For this review, use the dimensioned drawing (mm, ordinates from the lowest corner) and the shaded views. Coordinates: 2 decimals unless noted, no trailing zeros. Write each loop counter-clockwise with the first axis right and the second up, starting at its lowest first coordinate (ties: lowest second). Pieces come first, ordered by that corner, then holes. Notation, with made-up numbers: (-8.75, 46.5) - (44.25, 46.5) arc R21 ccw to (44.25, 64.5) - close; hole circle Ø8 at (81.5, 51). An arc over 180 degrees is marked (long way). Put each result on its own line as item: value.
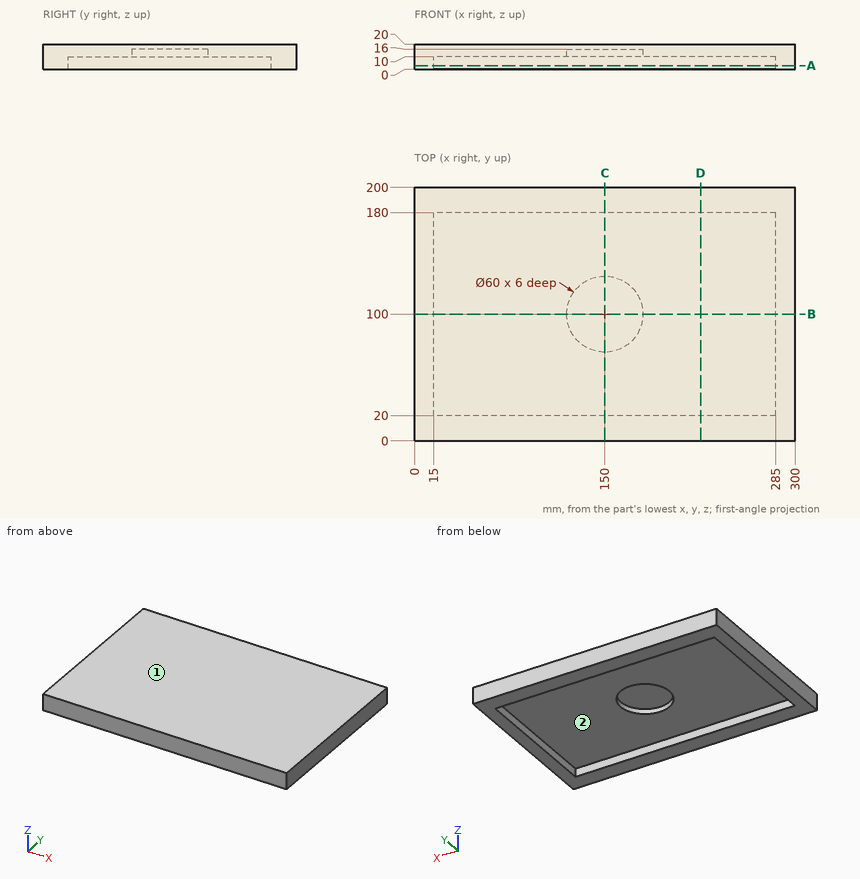
1. Consider section B-B on y = 100. State the section outline as (x, z) points, plus the area to 3 significant figures.
Determined:
outline: (0, 0) - (15, 0) - (15, 10) - (120, 10) - (120, 16) - (180, 16) - (180, 10) - (285, 10) - (285, 0) - (300, 0) - (300, 20) - (0, 20) - close
area: 2,940 mm^2
2. For pin 1 Ø12 at (x, y) = (162.5, 117.5) entering from -Z; pin 2 Ø3 at (x, y) = (263.5, 164.5) entering from -Z, all flat-tipped, find the tip position at first contact; note any pin that passes through.
Determined:
pin 1: stops at z = 16
pin 2: stops at z = 10
3. To check wall thickness, follow probe 1 along Y at (x, z) = (150, 14.5); probe 2 along Y at (x, z) = (167, 1); probe 3 along X at (y, z) = (65, 6.75). State the ranges of each line that lie inside material, in increasing order.
Determined:
probe 1: y = 0 to 70, 130 to 200
probe 2: y = 0 to 20, 180 to 200
probe 3: x = 0 to 15, 285 to 300
4. Consider section D-D on x = 225.5. State the section outline as (y, z) points.
Determined:
outline: (0, 0) - (20, 0) - (20, 10) - (180, 10) - (180, 0) - (200, 0) - (200, 20) - (0, 20) - close
5. The part is to be moulded in two halves that separate along X. For the marked faces 1 and 2, say which applies: +X half, -X half, draft (parallel to the pull), parting line (faces both ways), or undercut.
Determined:
face 1: draft
face 2: undercut
6. Consider section C-C on x = 150. State the section outline as (y, z) points.
Determined:
outline: (0, 0) - (20, 0) - (20, 10) - (70, 10) - (70, 16) - (130, 16) - (130, 10) - (180, 10) - (180, 0) - (200, 0) - (200, 20) - (0, 20) - close
7. Consider section A-A on z = 3. State the section outline as (x, y) points, plus the area to 3 significant figures.
Determined:
outline: (0, 0) - (300, 0) - (300, 200) - (0, 200) - close; hole (15, 20) - (285, 20) - (285, 180) - (15, 180) - close
area: 16,800 mm^2
